Could you check a few things on this model? Use its own coordinates, in mm. A direction names the side the tool comes from. Round coordinates to 2 decimals unless told otherwise and drop trailing zeros. Order: outer loops, then holes, each group sorted by start corner. A loop starts at its lowest first (then second) coordinate and runs counter-clockwise, first axis right, second up. Notation, with made-up numbers: (-14.5, 5) - (27.5, 5) arc R26 ccw to (27.5, 36) - close; hole circle Ø7 at (24, 31). An arc over 180 degrees is marked (long way). Use one line per item in the form item = value.
from build123d import *

# Parameters (mm, degrees)
SKETCH1_R           = 15
BOSS_EXTRUDE1_DEPTH = 257.5
SKETCH2_R           = 8
BOSS_EXTRUDE2_DEPTH = 50
BOSS_EXTRUDE3_START = 50
SKETCH3_R           = 8
BOSS_EXTRUDE3_DEPTH = 50


with BuildPart() as part:
    # Sketch1 → Boss-Extrude1 (new, symmetric)
    with BuildSketch(Plane.XY):
        Circle(SKETCH1_R)
    extrude(amount=BOSS_EXTRUDE1_DEPTH, both=True)

    # Sketch2 → Boss-Extrude2 (add)
    with BuildSketch(Plane.XY.offset(257.5)):
        Circle(SKETCH2_R)
    extrude(amount=BOSS_EXTRUDE2_DEPTH)

    # Sketch3 → Boss-Extrude3 (add)
    with BuildSketch(Plane(origin=(0, 0, -257.5), x_dir=(-1, 0, 0), z_dir=(0, 0, -1)).offset(BOSS_EXTRUDE3_START)):
        with Locations(Location((0, 0, 0), (0, 0, 180))):
            Circle(SKETCH3_R)
    extrude(amount=-BOSS_EXTRUDE3_DEPTH)


solid = part.part
Item 1: I need wall thicknesses on L1, parallel to Y at x = 0, z = 117; L2, parallel to Z at x = -11, y = 6.25; L3, parallel to Y at x = -12.75, z = -28. Which ranges of each line are inside material? Lowest first, please.
Found:
L1 = -15 to 15
L2 = -257.5 to 257.5
L3 = -7.9 to 7.9
Item 2: Imagine slicing it at C-C on z = 75. Please give me the cut outline in (x, y).
Found:
outline = circle Ø30 at (0, 0)
Item 3: If we mould it in two halves opening along X, with no side actions, what happens to faces 4 (the face through (-1.73, 7.81, -282.85)), 5 (the face through (0, 0, 307.5))? For each: released by +X, released by -X, zero draft, split by the parting line, or undercut.
Found:
face_4 = split by the parting line
face_5 = zero draft
Item 4: Will these pins go through, and if not, where does the flat tip stop? P1, Ø1.5, axis at x = -11.5, z = 0.5, coming from the -Y side; P2, Ø1.5, axis at x = 1, z = -129.5, coming from the +Y side; P3, Ø1, axis at y = 6.5, z = -7.5, coming from the +X side.
Found:
P1 = -10.46
P2 = 15
P3 = 13.75
Item 5: Imagine slicing it at A-A on y = 0. Please give me the cut outline in (x, z).
Found:
outline = (-15, -257.5) - (-8, -257.5) - (-8, -307.5) - (8, -307.5) - (8, -257.5) - (15, -257.5) - (15, 257.5) - (8, 257.5) - (8, 307.5) - (-8, 307.5) - (-8, 257.5) - (-15, 257.5) - close
Item 6: For faces 1 (the face through (6, -6, -257.5)), 2 (the face through (0, 0, -307.5)), 3 (the face through (-1.73, -7.81, 282.15)), which set-ups out of +Z, -Z, +X, -X, +Y, -Y let a thin tool reach every point of the face, with its end or its side?
Found:
face_1 = -Z
face_2 = -Z, +X, -X, +Y, -Y
face_3 = +Z
